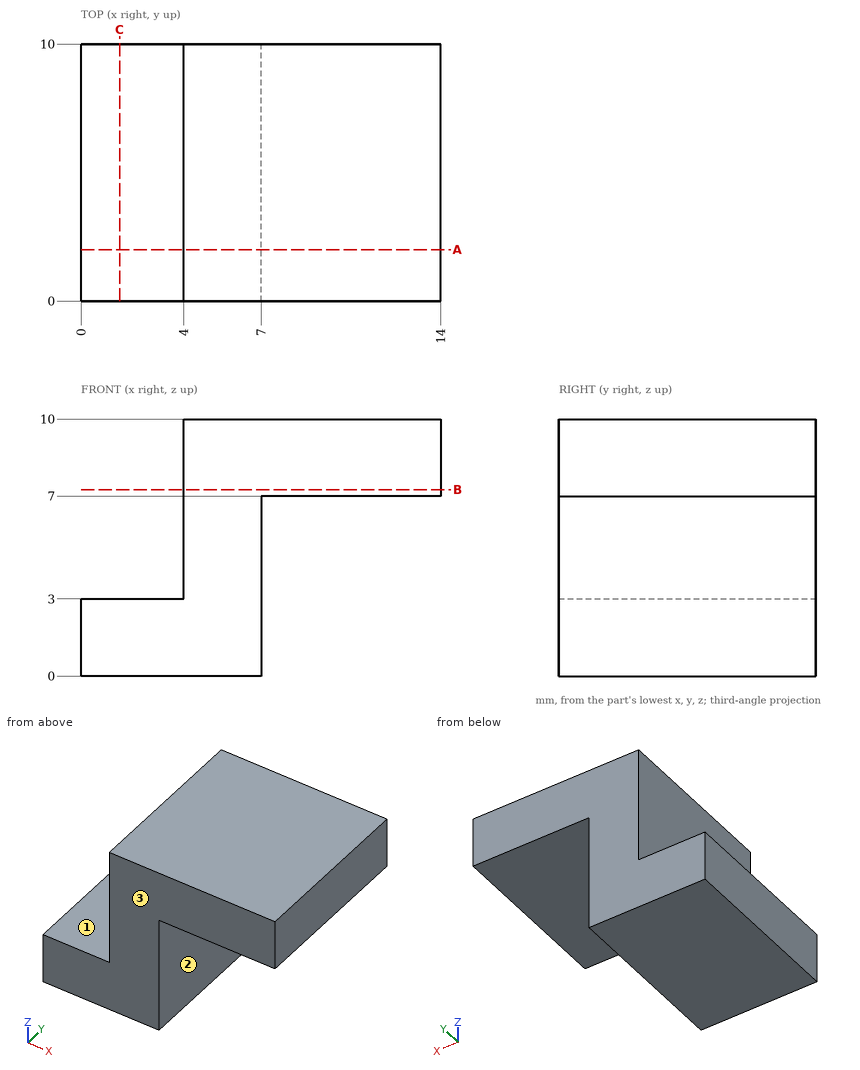
Geometry: see drawing. Coordinates: mm, zero at the bounding-box minimum. A direction names the side the tool comes from. Give positions to 0.01 mm unless a question says otherwise; leave off trailing zeros. Loops run counter-clockwise (first coordinate to the right, second up) from the corner with the lowest first, then second, coordinate; pieces in that order, holes last. Notation, with made-up numbers: M 55.25,43.25 L 108.25,43.25 A22 cw 108.25,65.25 Z; hole C 40.25,9.5 d1. An arc over 180 degrees is marked long. Use one line per item in the form item = value.
1. Section query B-B, the plane z = 7.25. Return the cut outline in (x, y), and give its area (3 significant figures).
Numbers:
outline = M 4,0 L 14,0 L 14,10 L 4,10 Z
area = 100 mm²
2. Line query: L1, parallel to Z at x = 12.5, y = 5; L2, parallel to X at y = 6, z = 2; L3, parallel to X at y = 6.75, z = 6.75. Output: solid intervals per line, ascending.
Numbers:
L1 = 7 to 10
L2 = 0 to 7
L3 = 4 to 7
3. First-contact query: pin 1 (5 mm diameter, centred on x = 1.5, z = 3, fed in from -Y); pin 2 (1 mm diameter, centred on y = 4.5, z = 6.5, fed in from -X); pin 3 (2 mm diameter, centred on x = 11, y = 6.5, fed in from -Z); pin 4 (1.2 mm diameter, centred on x = 2.5, y = 7.5, fed in from +Z). Flat tips, straight axial feed; report the tip coordinate or a pass-through.
Numbers:
pin_1 = 0
pin_2 = 4
pin_3 = 7
pin_4 = 3
4. Section query A-A, the plane y = 2. Return the cut outline in (x, z).
Numbers:
outline = M 0,0 L 7,0 L 7,7 L 14,7 L 14,10 L 4,10 L 4,3 L 0,3 Z
5. Section query C-C, the plane x = 1.5. Return the cut outline in (y, z).
Numbers:
outline = M 0,0 L 10,0 L 10,3 L 0,3 Z
6. Reachability of the marked faces 1, 2 and 3 from +Z, -Z, +X, -X, +Y, -Y: full face, straight path, thin tool, end or side. Return the list, or none.
Numbers:
face_1 = +Z, -X, +Y, -Y
face_2 = -Z, +X, +Y, -Y
face_3 = +Z, -Z, +X, -X, -Y
